```python
from build123d import *

# Parameters (mm, degrees)
SKETCH_1_W           = 200
SKETCH_1_H           = 150
BOSS_EXTRUDE_1_DEPTH = 30
SKETCH_2_R           = 25
BOSS_EXTRUDE_2_DEPTH = 30
SKETCH_4_W           = 15
SKETCH_4_H           = 80
BOSS_EXTRUDE_3_DEPTH = 50


with BuildPart() as part:
    # Sketch 1 → Boss-Extrude 1 (new body)
    with BuildSketch(Plane(origin=(0, 0, 0), x_dir=(1, 0, 0), z_dir=(0, 1, 0))):
        Rectangle(SKETCH_1_W, SKETCH_1_H)
    extrude(amount=BOSS_EXTRUDE_1_DEPTH)

    # Sketch 2 → Boss-Extrude 2 (add)
    with BuildSketch(Plane.XY.offset(75)):
        with BuildLine():
            Line((-55.814702058, 142.01633562), (-100, 30))
            Line((-100, 30), (100, 30))
            Line((100, 30), (55.814702058, 142.01633562))
            ThreePointArc((55.814702058, 142.01633562), (0, 180), (-55.814702058, 142.01633562))
        make_face()
        with Locations((0, 120)):
            Circle(SKETCH_2_R, mode=Mode.SUBTRACT)
    boss_extrude_2 = extrude(amount=-BOSS_EXTRUDE_2_DEPTH)

    # Sketch 4 → Boss-Extrude 3 (add)
    with BuildSketch(Plane.XY.offset(75)):
        with Locations((0, 40)):
            Rectangle(SKETCH_4_W, SKETCH_4_H)
    boss_extrude_3 = extrude(amount=BOSS_EXTRUDE_3_DEPTH)

    # Mirror 1: Boss-Extrude 2, Boss-Extrude 3 across plane
    add(boss_extrude_2.mirror(Plane.XY))
    add(boss_extrude_3.mirror(Plane.XY))


solid = part.part
```
The listing builds one solid part. Answer for the finished solid, in the listing's coordinates (mm). A direction names the side the tool comes from. Round coordinates to 2 decimals unless told otherwise and drop trailing zeros. Loops run counter-clockwise (first coordinate to the right, second up) from the corner with the lowest first, then second, coordinate; pieces in that order, holes last. Notation, with made-up numbers: (47, 16.5) -> (53, 16.5) arc R27 ccw to (53, 34.5) -> close; hole circle Ø2 at (83, 54.25). An arc over 180 degrees is marked (long way). Use one line per item in the form item = value.
1. A tool of negligible diameter and unlimited length cuts with its end or side. For faces 1 (the flat face through (-7.5, 39, -100)), 2 (the flat face through (0, 80, 100)), 3 (the flat face through (0, 80, -100)), 4 (the flat face through (-7.5, 39, 100)), from which of +Z, -Z, +X, -X, +Y, -Y can it reach the whole face along a straight path? Write none if from no direction.
Answer key:
face_1 = -Z, -X, +Y, -Y
face_2 = +Z, +X, -X, +Y
face_3 = -Z, +X, -X, +Y
face_4 = +Z, -X, +Y, -Y
2. Find the intervals of material crossed by probe 1 along Z at (x, y) = (3, 71); probe 2 along Z at (x, y) = (34, 42); probe 3 along Y at (x, z) = (4, 78), in increasing order. Write a range as [from, to].
Answer key:
probe_1 = [-125, -45], [45, 125]
probe_2 = [-75, -45], [45, 75]
probe_3 = [0, 80]
3. For a pull along Z with two mould halves and no side action, classify faces 5 (the flat face through (7.5, 39, -100)), 6 (the flat face through (0, 41, -125)), 7 (the flat face through (-1, 89, 45)), 8 (the flat face through (-1, 30, -1)) as released by +Z, released by -Z, zero draft, split by the parting line, or undercut.
Answer key:
face_5 = zero draft
face_6 = released by -Z
face_7 = undercut
face_8 = undercut
4. The part is cut by section D-D on z = -91. Determine the outline of the cut face in (x, y), and give its area (3 significant figures).
Answer key:
outline = (-7.5, 0) -> (7.5, 0) -> (7.5, 80) -> (-7.5, 80) -> close
area = 1,200 mm²
5. The part is cut by section B-B on y = 36.5. Determine the outline of the cut face in (x, z), and give its area (3 significant figures).
Answer key:
outline = (-97.44, -75) -> (-7.5, -75) -> (-7.5, -125) -> (7.5, -125) -> (7.5, -75) -> (97.44, -75) -> (97.44, -45) -> (-97.44, -45) -> close; (-97.44, 45) -> (97.44, 45) -> (97.44, 75) -> (7.5, 75) -> (7.5, 125) -> (-7.5, 125) -> (-7.5, 75) -> (-97.44, 75) -> close
area = 13,200 mm²
6. Flat-ended cylindrical pins translate along their axes: pin 1 Ø8 at (x, z) = (-18, 74.5) entering from +Y; pin 2 Ø12 at (y, z) = (72, 94.5) entering from +X; pin 3 Ø10 at (y, z) = (31.5, 59) entering from -X; pin 4 Ø12 at (x, z) = (-2, 107.5) entering from +Y. Find the tip coordinate at first contact, or state that the pin passes through.
Answer key:
pin_1 = 178.34
pin_2 = 7.5
pin_3 = -100
pin_4 = 80
7. The part is cut by section C-C on y = 120. Determine the outline of the cut face in (x, z).
Answer key:
outline = (-64.5, -75) -> (-25, -75) -> (-25, -45) -> (-64.5, -45) -> close; (-64.5, 45) -> (-25, 45) -> (-25, 75) -> (-64.5, 75) -> close; (25, -75) -> (64.5, -75) -> (64.5, -45) -> (25, -45) -> close; (25, 45) -> (64.5, 45) -> (64.5, 75) -> (25, 75) -> close
8. The part is cut by section A-A on x = 0. Determine the outline of the cut face in (y, z).
Answer key:
outline = (0, -125) -> (80, -125) -> (80, -75) -> (95, -75) -> (95, -45) -> (30, -45) -> (30, 45) -> (95, 45) -> (95, 75) -> (80, 75) -> (80, 125) -> (0, 125) -> close; (145, -75) -> (180, -75) -> (180, -45) -> (145, -45) -> close; (145, 45) -> (180, 45) -> (180, 75) -> (145, 75) -> close
